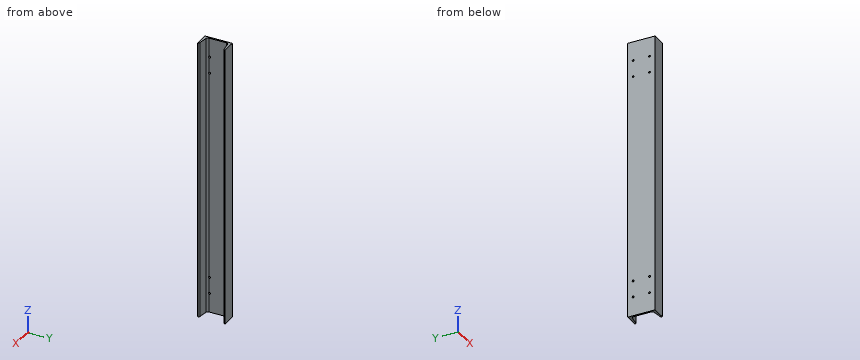
```python
from build123d import *

# Parameters (mm, degrees)
BOSS_EXTRUDE1_DEPTH   = 1022
M8_TAPPED_HOLE1_D     = 6.8
M8_TAPPED_HOLE1_DEPTH = 19.75
M8_TAPPED_HOLE1_TIP   = 2.042926105


with BuildPart() as part:
    # Sketch1 → Boss-Extrude1 (new body)
    with BuildSketch(Plane.XY):
        with BuildLine():
            Line((0, 0), (-50, 0))
            Line((-50, 0), (-50, -100))
            Line((-50, -100), (0, -100))
            Line((0, -100), (0, -98.925311188))
            ThreePointArc((0, -98.925311188), (-1.103806889, -95.973045557), (-3.873721046, -94.469104878))
            Line((-3.873721046, -94.469104878), (-36.682971358, -89.858065454))
            ThreePointArc((-36.682971358, -89.858065454), (-41.915031432, -87.017288616), (-44, -81.440786869))
            Line((-44, -81.440786869), (-44, -18.559213131))
            ThreePointArc((-44, -18.559213131), (-41.915031432, -12.982711384), (-36.682971358, -10.141934546))
            Line((-36.682971358, -10.141934546), (-3.873721046, -5.530895122))
            ThreePointArc((-3.873721046, -5.530895122), (-1.103806889, -4.026954443), (0, -1.074688812))
            Line((0, -1.074688812), (0, 0))
        make_face()
    extrude(amount=BOSS_EXTRUDE1_DEPTH)

    # M8 Tapped Hole1
    with Locations(Plane.ZY.offset(50)):
        with Locations((70, -20), (130, -20), (130, -80), (70, -80), (892, -20), (952, -20), (952, -80), (892, -80)):
            Hole(M8_TAPPED_HOLE1_D / 2, depth=M8_TAPPED_HOLE1_DEPTH)
            with Locations((0, 0, -(M8_TAPPED_HOLE1_DEPTH + M8_TAPPED_HOLE1_TIP / 2))):  # 118° drill point
                Cone(0, M8_TAPPED_HOLE1_D / 2, M8_TAPPED_HOLE1_TIP, mode=Mode.SUBTRACT)


solid = part.part
```
Geometry: final body of the model. Coordinates: model frame, mm. Give positions to 0.01 mm unless a question says otherwise; leave off trailing zeros. Write each loop counter-clockwise with the first axis right and the second up, starting at its lowest first coordinate (ties: lowest second). Pieces come first, ordered by that corner, then holes.
1. Line query: probe 1 along Z at (x, y) = (-45.25, -20); probe 2 along Y at (x, z) = (-45.75, 70); probe 3 along X at (y, z) = (-81.5, 533.5). Output: solid intervals per line, ascending.
2. Pin query (flat end, axial travel): P1, Ø2, axis at x = -18, z = 229, coming from the +Y side; P2, Ø5, axis at y = -32, z = 622.5, coming from the +X side. Return the tip coordinate at first contact, or that it passes through.
3. Section query C-C, the plane y = -67. Return loops of the section in (x, z).
4. Section query A-A, the plane z = 144. Return loops of the section in (x, y).
5. Section query B-B, the plane x = -14. Return loops of the section in (y, z), then the cut area to 3 significant figures.
Computed:
1. probe 1: z = 0 to 66.6, 73.4 to 126.6, 133.4 to 888.6, 895.4 to 948.6, 955.4 to 1022
1. probe 2: y = -100 to -83.4, -76.6 to -23.4, -16.6 to 0
1. probe 3: x = -50 to -44
2. P1: stops at y = 0
2. P2: stops at x = -44
3. outline: (-50, 0) - (-44, 0) - (-44, 1022) - (-50, 1022) - close
4. outline: (-50, -100) - (0, -100) - (0, -98.93) arc R4.5 ccw to (-3.87, -94.47) - (-36.68, -89.86) arc R8.5 cw to (-44, -81.44) - (-44, -18.56) arc R8.5 cw to (-36.68, -10.14) - (-3.87, -5.53) arc R4.5 ccw to (0, -1.07) - (0, 0) - (-50, 0) - close
5. outline: (-100, 0) - (-93.05, 0) - (-93.05, 1022) - (-100, 1022) - close; (-6.95, 0) - (0, 0) - (0, 1022) - (-6.95, 1022) - close
5. area: 14,200 mm2
